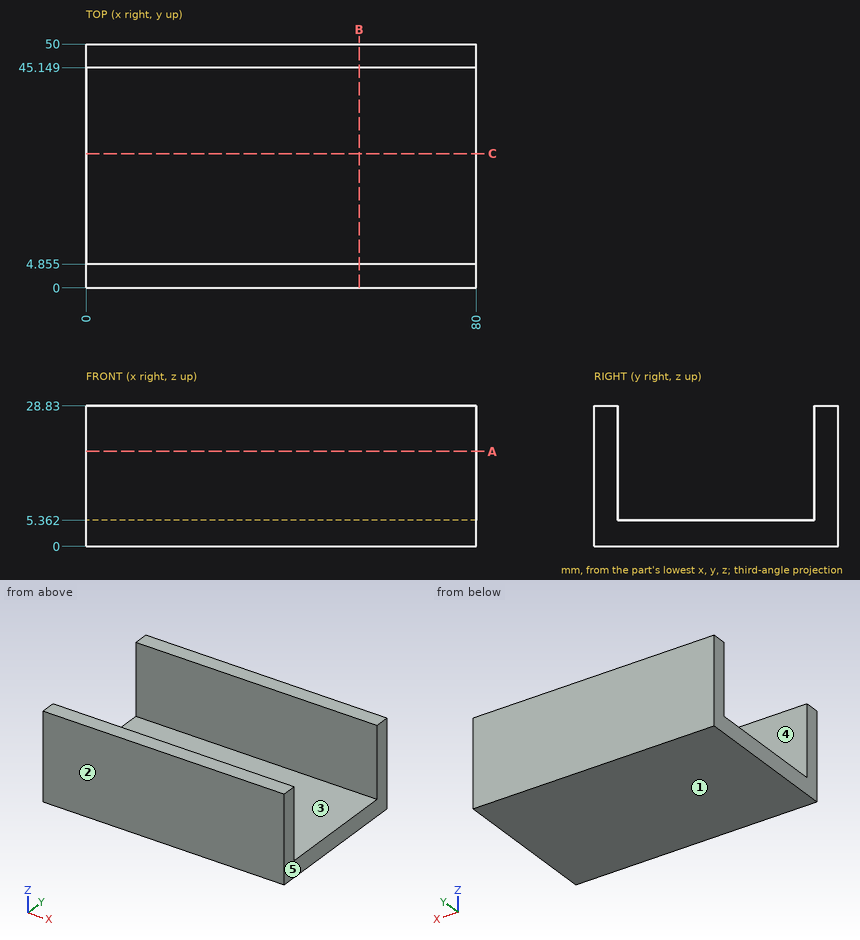
Study the drawing (mm; zero at the part's minimum x, y, z) and answer. A direction names the side the tool comes from. Coordinates: 2 decimals unless noted, no trailing zeros. Write each loop counter-clockwise with the first axis right and the second up, starting at its lowest first coordinate (ties: lowest second). Pieces come first, ordered by that corner, then holes. Notation, with made-up numbers: (82, -11.75) - (128, -11.75) arc R31 cw to (128, 25.25) - close; hole circle Ø4 at (89.25, 44). An arc over 180 degrees is marked (long way). Return JSON: item names as keys, results as strings. Group by question number.
1. Given pin 1 (20 mm diameter, centred on x = 30.5, y = 25.5, fed in from +Z), flat-ended and moving along its own axis, determine where the tip first touches the part or whether it passes through.
2. A cutting plane is placed at A-A, the plane z = 19.5. Determine the outline of the cut face in (x, y) (1 decimal).
3. Which of the six approach directions +Z, -Z, +X, -X, +Y, -Y give full straight-line access (tool end or side, diameter ignored) to the marked faces 4 and 5?
4. A cutting plane is placed at B-B, the plane x = 56. Determine the outline of the cut face in (y, z) (1 decimal).
5. A cutting plane is placed at C-C, the plane y = 27.5. Determine the outline of the cut face in (x, z), plus the area to 3 significant figures.
6. Determine the mould class of the marked faces 1, 2 and 3 for opening direction Y: released by +Y, released by -Y, zero draft, split by the parting line, or undercut.
7. Straight lines are drawn through the part: L1, parallel to Y at x = 23.5, z = 13.5 (1 decimal); L2, parallel to Z at x = 52, y = 29. For each, find the intervals that lie inside material, in ascending order.
Ans:
{
 "1": {"pin 1": "z = 5.36"},
 "2": {"outline": "(0, 0) - (80, 0) - (80, 4.9) - (0, 4.9) - close; (0, 45.1) - (80, 45.1) - (80, 50) - (0, 50) - close"},
 "3": {"face 4": "+Z, +X, -X", "face 5": "+Z, -Z, +X, +Y, -Y"},
 "4": {"outline": "(0, 0) - (50, 0) - (50, 28.8) - (45.1, 28.8) - (45.1, 5.4) - (4.9, 5.4) - (4.9, 28.8) - (0, 28.8) - close"},
 "5": {"outline": "(0, 0) - (80, 0) - (80, 5.36) - (0, 5.36) - close", "area": "429 mm²"},
 "6": {"face 1": "zero draft", "face 2": "released by -Y", "face 3": "undercut"},
 "7": {"L1": "0 to 4.9, 45.1 to 50", "L2": "0 to 5.36"}
}
